Source: CAD feature listing. Evaluate the final solid. Frame: model axes, mm. A direction names the side the tool comes from. Give positions to 0.01 mm unless a question says otherwise; leave off trailing zeros. Write each loop counter-clockwise with the first axis right and the second up, starting at its lowest first coordinate (ties: lowest second). Pieces come first, ordered by that corner, then holes. Notation, with made-up numbers: (42, 71.25) -> (58, 71.25) arc R6 ccw to (58, 79.25) -> close; hole circle Ø2 at (-25.5, 7). An arc over 180 degrees is marked (long way). Use one line per item in the form item = value. Start each with the question number.
(1) Cut plane B-B, the plane y = 10.5. Output: boundary loops of the cut face in (x, z), and give its area (3 significant figures).
(2) Material intervals for line 1 along Y through (x, z) = (-102, 13); line 2 along Y through (x, z) = (-87, 113.5); line 3 along Y through (x, z) = (-26, 137), sorted ascending. Write a range as from..to.
(3) Draft query along Y for faces 1 (the face through (57.914, 139.816, 308.188)), 2 (the face through (-20, 147, 310)), 3 (the face through (-91.696, -134.119, 151.844)), 4 (the face through (-111, -90, 308)). Return one class per face: pulls with the +Y half, pulls with the -Y half, needs draft (parallel to the pull), parting line crosses it, or undercut.
(4) Cut plane A-A, the plane z = 58. Output: boundary loops of the cut face in (x, y), and give its area (3 significant figures).
(5) First-contact query: P1, Ø2, axis at y = -100, z = 165, coming from the +X side; P2, Ø2, axis at y = 121.5, z = 40, coming from the +X side; P3, Ø9.5, axis at x = -46.19, y = 136.19, coming from the -Z side. Flat tips, straight axial feed; report the tip coordinate or a pass-through.
(6) Set-up query: faces 5 (the face through (26.387, 136.276, 309.014)), 6 (the face through (-32.85, 133.6, 309.01)), 7 (the face through (-78.43, -114.72, 309.01)), 8 (the face through (-147.25, -59.99, 151.84)), 9 (the face through (30.85, 159.32, 151.84)). Return all of +Z, -Z, +X, -X, +Y, -Y with unobstructed straight access to the full face (end or side cutting, diameter ignored); none if empty.
from build123d import *

# Parameters (mm, degrees)
BOSS_EXTRUDE1_DEPTH   = 310
SHELL1_T              = -2
CUT_EXTRUDE1_DEPTH    = 10
CUT_EXTRUDE2_DEPTH    = 397.026111511
CUT_EXTRUDE3_DEPTH    = 5
SKETCH5_R             = 3
CUT_EXTRUDE4_DEPTH    = 10
SKETCH10_R            = 3
BOSS_EXTRUDE3_DEPTH   = 2
M3_TAPPED_HOLE1_D     = 2.5
M3_TAPPED_HOLE1_DEPTH = 4
CUT_EXTRUDE5_REACH    = 492.141
SKETCH17_W            = 3.5
SKETCH17_H            = 301


with BuildPart() as part:
    # Sketch1 → Boss-Extrude1 (new body)
    with BuildSketch(Plane.XY):
        Polygon((-174.265144247, 0), (-123.224065222, -123.224065222), (0, -174.265144247), (123.224065222, -123.224065222), (174.265144247, 0), (123.224065222, 123.224065222), (0, 174.265144247), (-123.224065222, 123.224065222), align=None)
    extrude(amount=BOSS_EXTRUDE1_DEPTH)

    # Shell1
    shell1_openings = [part.faces().sort_by_distance(p)[0] for p in [
        (0, 0, 0),
    ]]
    offset(amount=SHELL1_T, openings=shell1_openings, kind=Kind.INTERSECTION)

    # Sketch2 → Cut-Extrude1 (cut)
    with BuildSketch(Plane.XY.offset(310)):
        Polygon((104.089893603, 104.089893603), (0, 147.20533924), (-104.089893603, 104.089893603), (-147.20533924, 0), (-104.089893603, -104.089893603), (0, -147.20533924), (104.089893603, -104.089893603), (147.20533924, 0), align=None)
    extrude(amount=-CUT_EXTRUDE1_DEPTH, mode=Mode.SUBTRACT)

    # Sketch3 → Cut-Extrude2 (cut, through all)
    with BuildSketch(Plane.XY.offset(310)):
        Polygon((70.138181093, 169.328548035), (-63.801020235, -154.029288344), (130.028007017, -234.315900213), (263.967208344, 89.041936166), align=None)
    extrude(amount=-CUT_EXTRUDE2_DEPTH, mode=Mode.SUBTRACT)

    # Sketch4 → Cut-Extrude3 (cut)
    with BuildSketch(Plane.XY.offset(310)):
        Polygon((-143.932898959, 151.622295845), (-51.544945707, 113.353952609), (-116.60112921, -43.705567918), (-208.989082461, -5.437224682), align=None)
    extrude(amount=-CUT_EXTRUDE3_DEPTH, mode=Mode.SUBTRACT)

    # Sketch5 → Cut-Extrude4 (cut)
    with BuildSketch(Plane.XY.offset(310)):
        with Locations((0, 155.323280742)):
            Circle(SKETCH5_R)
        with Locations((-46.193976626, 136.189109124)):
            Circle(SKETCH5_R)
        with Locations((46.193976626, 136.189109124)):
            Circle(SKETCH5_R)
        with Locations((-128.964316707, -63.636168463)):
            Circle(SKETCH5_R)
        with Locations((-109.830145089, -109.830145089)):
            Circle(SKETCH5_R)
        with Locations((-63.636168463, -128.964316707)):
            Circle(SKETCH5_R)
    extrude(amount=-CUT_EXTRUDE4_DEPTH, mode=Mode.SUBTRACT)

    # Sketch10 → Boss-Extrude3 (add)
    with BuildSketch(Plane(origin=(-60.846665746, -146.896845669, 0), x_dir=(0.9238795325112958, -0.3826834323650679, 0), z_dir=(0.3826834323650679, 0.9238795325112958, 0))):
        with Locations(Location((-9.5, -280, 0), (0, 0, 180))):
            Circle(SKETCH10_R)
        with Locations(Location((-9.5, -266.5, 0), (0, 0, 180))):
            Circle(SKETCH10_R)
        with Locations(Location((-9.5, -33.5, 0), (0, 0, 180))):
            Circle(SKETCH10_R)
        with Locations(Location((-9.5, -20, 0), (0, 0, 180))):
            Circle(SKETCH10_R)
    extrude(amount=BOSS_EXTRUDE3_DEPTH)

    # M3 Tapped Hole1
    with Locations(Plane(origin=(-61.612032611, -148.744604734, 0), x_dir=(-0.9238795325112958, 0.3826834323650679, 0), z_dir=(-0.3826834323650679, -0.9238795325112958, 0))):
        with Locations((9.5, -280), (9.5, -266.5), (9.5, -33.5), (9.5, -20)):
            Hole(M3_TAPPED_HOLE1_D / 2, depth=M3_TAPPED_HOLE1_DEPTH)

    # Sketch17 → Cut-Extrude5 (cut, up to next)
    with BuildSketch(Plane(origin=(61.612032611, 148.744604734, 0), x_dir=(0.923879532511296, -0.38268343236506785, 0), z_dir=(0.38268343236506785, 0.923879532511296, 0)), mode=Mode.PRIVATE) as cut_extrude5_sk1:
        with Locations((-1.75, -150.5)):
            Rectangle(SKETCH17_W, SKETCH17_H)
    cut_extrude5_tool1 = extrude(cut_extrude5_sk1.sketch, amount=-CUT_EXTRUDE5_REACH, mode=Mode.PRIVATE) & part.part
    add(cut_extrude5_tool1.solids().sort_by_distance((59.995243, 149.414301, 150.5))[0], mode=Mode.SUBTRACT)


solid = part.part
Geometry says:
q1.outline = (-169.92, 0) -> (-167.75, 0) -> (-167.75, 305) -> (-169.92, 305) -> close
q1.area = 660 mm^2
q2.line_1 = -132.02..-129.85, 129.85..132.02
q2.line_2 = -138.23..-136.06, 136.06..138.23
q2.line_3 = 161.33..163.5
q3.face_1 = pulls with the -Y half
q3.face_2 = needs draft
q3.face_3 = undercut
q3.face_4 = undercut
q4.outline = (-174.27, 0) -> (-123.22, -123.22) -> (-61.61, -148.74) -> (-60.85, -146.9) -> (-121.69, -121.69) -> (-172.1, 0) -> (-121.69, 121.69) -> (0, 172.1) -> (57.61, 148.24) -> (58.38, 150.08) -> (0, 174.27) -> (-123.22, 123.22) -> close
q4.area = 1,050 mm^2
q5.P1 = -130.26
q5.P2 = -119.75
q5.P3 = 308
q6.face_5 = +Z, -Z, -Y
q6.face_6 = +Z, -Z
q6.face_7 = +Z, -Z, +X
q6.face_8 = -Z, +X
q6.face_9 = -Z, -Y
